from build123d import *

# Parameters (mm, degrees)
SKETCH_1_W                = 160
SKETCH_1_H                = 64
EXTRUDE_1_DEPTH           = 19
FILLET_1_R                = 10
HOLE_WIZARD_M6_1_D        = 5
HOLE_WIZARD_2_D           = 6.6
HOLE_WIZARD_2_CSINK_D     = 12.8
HOLE_WIZARD_2_CSINK_ANGLE = 90


with BuildPart() as part:
    # 草图1 → 凸台-拉伸1 (new body)
    with BuildSketch(Plane.XY):
        Rectangle(SKETCH_1_W, SKETCH_1_H)
    extrude(amount=EXTRUDE_1_DEPTH)

    # 圆角1
    fillet_1_edges = [part.edges().sort_by_distance(p)[0] for p in [
        (80, -32, 9.5),
        (-80, -32, 9.5),
        (-80, 32, 9.5),
        (80, 32, 9.5),
    ]]
    fillet(fillet_1_edges, radius=FILLET_1_R)

    # M6 螺纹孔1 (through all)
    with Locations(Plane.XY.offset(19)):
        with Locations((-60, 25), (-60, -25), (47, 25), (47, -25)):
            Hole(HOLE_WIZARD_M6_1_D / 2)

    # 打孔尺寸(%根据)内六角花形半沉头螺钉的类型2 (through all)
    with Locations(Plane(origin=(0, 0, 0), x_dir=(-1, 0, 0), z_dir=(0, 0, -1))):
        with Locations((-52, 0), (8, 0)):
            CounterSinkHole(HOLE_WIZARD_2_D / 2, HOLE_WIZARD_2_CSINK_D / 2, counter_sink_angle=HOLE_WIZARD_2_CSINK_ANGLE)


solid = part.part
Input: part model. Units: mm. Frame: model coordinates. Coordinates: 2 decimals unless noted, no trailing zeros. Loops run counter-clockwise (first coordinate to the right, second up) from the corner with the lowest first, then second, coordinate; pieces in that order, holes last. Notation, with made-up numbers: (76, 80.25) -> (110, 80.25) arc R32 ccw to (110, 112.25) -> close; hole circle Ø4 at (4.25, -32). An arc over 180 degrees is marked (long way). One line per item, written item: value.
(1) Cut plane C-C (y = 0). Output: boundary loops of the cut face in (x, z), then the cut area to 3 significant figures.
Answer below:
outline: (-80, 0) -> (-14.4, 0) -> (-11.3, 3.1) -> (-11.3, 19) -> (-80, 19) -> close; (-4.7, 3.1) -> (-1.6, 0) -> (45.6, 0) -> (48.7, 3.1) -> (48.7, 19) -> (-4.7, 19) -> close; (55.3, 3.1) -> (58.4, 0) -> (80, 0) -> (80, 19) -> (55.3, 19) -> close
area: 2,770 mm2
(2) Cut plane A-A (x = -8). Output: boundary loops of the cut face in (y, z).
Answer below:
outline: (-32, 0) -> (-6.4, 0) -> (-3.3, 3.1) -> (-3.3, 19) -> (-32, 19) -> close; (3.3, 3.1) -> (6.4, 0) -> (32, 0) -> (32, 19) -> (3.3, 19) -> close
(3) Ray query, line 1 along X through (y, z) = (0, 12.5); line 2 along Y through (x, z) = (-60, 8.75); line 3 along X through (y, z) = (26, 5). Return the intervals inside material, ascending.
Answer below:
line 1: x = -80 to -11.3, -4.7 to 48.7, 55.3 to 80
line 2: y = -32 to -27.5, -22.5 to 22.5, 27.5 to 32
line 3: x = -79.17 to -62.29, -57.71 to 44.71, 49.29 to 79.17
(4) Cut plane D-D (z = 17.5). Output: boundary loops of the cut face in (x, y), then the cut area to 3 significant figures.
Answer below:
outline: (-80, -22) arc R10 ccw to (-70, -32) -> (70, -32) arc R10 ccw to (80, -22) -> (80, 22) arc R10 ccw to (70, 32) -> (-70, 32) arc R10 ccw to (-80, 22) -> close; hole circle Ø5 at (-60, -25); hole circle Ø5 at (-60, 25); hole circle Ø6.6 at (-8, 0); hole circle Ø5 at (47, -25); hole circle Ø5 at (47, 25); hole circle Ø6.6 at (52, 0)
area: 10,000 mm2
(5) Pin query (flat end, axial travel): pin 1 Ø1 at (y, z) = (-24.5, 14.5) entering from -X. Return the tip coordinate at first contact, or that it passes through.
Answer below:
pin 1: stops at x = -79.8
(6) Cut plane B-B (x = -60). Output: boundary loops of the cut face in (y, z), then the cut area to 3 significant figures.
Answer below:
outline: (-32, 0) -> (-27.5, 0) -> (-27.5, 19) -> (-32, 19) -> close; (-22.5, 0) -> (22.5, 0) -> (22.5, 19) -> (-22.5, 19) -> close; (27.5, 0) -> (32, 0) -> (32, 19) -> (27.5, 19) -> close
area: 1,030 mm2
(7) Draft query along X for faces 1 (the face through (80, 0, 9)), 2 (the face through (45.66, 27.11, 9.37)), 3 (the face through (-1, 32, 9)). Return one class per face: pulls with the +X half, pulls with the -X half, needs draft (parallel to the pull), parting line crosses it, or undercut.
Answer below:
face 1: pulls with the +X half
face 2: undercut
face 3: needs draft
